Design review of the part built by this model. Coordinates are the model's own, in mm. A direction names the side the tool comes from. Round coordinates to 2 decimals unless told otherwise and drop trailing zeros. Order: outer loops, then holes, each group sorted by start corner. A loop starts at its lowest first (then second) coordinate and runs counter-clockwise, first axis right, second up. Notation, with made-up numbers: (39.5, 73) - (44.5, 73) arc R11 cw to (44.5, 93) - close; hole circle Ø4 at (89, 70). An arc over 180 degrees is marked (long way). Write item = value, one per line.
from build123d import *

# Parameters (mm, degrees)
SKETCH_1_W                = 380
SKETCH_1_H                = 270
EXTRUDE_1_DEPTH           = 7.5
CHAMFER_1_SIZE            = 1
SKETCH_2_R                = 20
CUT_EXTRUDE_1_DEPTH       = 15
HOLE_WIZARD_3_D           = 6.6
HOLE_WIZARD_3_CBORE_D     = 11
HOLE_WIZARD_3_CBORE_DEPTH = 6.8
SKETCH_9_R                = 5.5
CUT_EXTRUDE_2_DEPTH       = 234.559414283
SKETCH_11_R               = 52.5
CUT_EXTRUDE_3_DEPTH       = 4
HOLE_WIZARD_M6_1_D        = 5
SKETCH_15_R               = 3
CUT_EXTRUDE_4_DEPTH       = 9


with BuildPart() as part:
    # 草图1 → 凸台-拉伸1 (new, symmetric)
    with BuildSketch(Plane(origin=(0, 0, 0), x_dir=(1, 0, 0), z_dir=(0, 1, 0))):
        Rectangle(SKETCH_1_W, SKETCH_1_H)
    extrude(amount=EXTRUDE_1_DEPTH, both=True)

    # 倒角1
    chamfer_1_edges = [part.edges().sort_by_distance(p)[0] for p in [
        (190, 0, 135),
        (-190, 0, 135),
        (-190, 0, -135),
        (190, 0, -135),
    ]]
    chamfer(chamfer_1_edges, length=CHAMFER_1_SIZE)

    # 草图2 → 切除-拉伸1 (cut)
    with BuildSketch(Plane(origin=(0, 7.5, 0), x_dir=(1, 0, 0), z_dir=(0, 1, 0))):
        with Locations(Location((0, 0, 0), (0, 0, 270))):
            Circle(SKETCH_2_R)
    extrude(amount=-CUT_EXTRUDE_1_DEPTH, mode=Mode.SUBTRACT)

    # 打孔尺寸(%根据)内六角圆柱头螺钉的类型3 (through all)
    with Locations(Plane(origin=(0, 7.5, 0), x_dir=(1, 0, 0), z_dir=(0, 1, 0))):
        with Locations((-175, 120), (-60, 120), (-60, -120), (-175, 0), (-175, -120), (175, -120), (175, 0), (60, -120), (60, 120), (175, 120)):
            CounterBoreHole(HOLE_WIZARD_3_D / 2, HOLE_WIZARD_3_CBORE_D / 2, HOLE_WIZARD_3_CBORE_DEPTH)

    # 草图9 → 切除-拉伸2 (cut, through all)
    with BuildSketch(Plane(origin=(0, 7.5, 0), x_dir=(1, 0, 0), z_dir=(0, 1, 0))):
        with Locations(Location((-29.489473594, 20.648751709, 0), (0, 0, 270))):
            Circle(SKETCH_9_R)
        with Locations(Location((-29.489473594, -20.648751709, 0), (0, 0, 270))):
            Circle(SKETCH_9_R)
        with Locations(Location((-32.5, 0, 0), (0, 0, 270))):
            Circle(SKETCH_9_R)
        with Locations(Location((29.489473594, -20.648751709, 0), (0, 0, 90))):
            Circle(SKETCH_9_R)
        with Locations(Location((32.5, 0, 0), (0, 0, 90))):
            Circle(SKETCH_9_R)
        with Locations(Location((29.489473594, 20.648751709, 0), (0, 0, 90))):
            Circle(SKETCH_9_R)
    extrude(amount=-CUT_EXTRUDE_2_DEPTH, mode=Mode.SUBTRACT)

    # 草图11 → 切除-拉伸3 (cut)
    with BuildSketch(Plane(origin=(0, 7.5, 0), x_dir=(1, 0, 0), z_dir=(0, 1, 0))):
        with Locations(Location((0, 0, 0), (0, 0, 270))):
            Circle(SKETCH_11_R)
    extrude(amount=-CUT_EXTRUDE_3_DEPTH, mode=Mode.SUBTRACT)

    # M6 螺纹孔1 (through all)
    with Locations(Plane(origin=(0, 7.5, 0), x_dir=(1, 0, 0), z_dir=(0, 1, 0))):
        with Locations((122.5, -7), (122.5, 23), (-122.5, 23), (-122.5, -7)):
            Hole(HOLE_WIZARD_M6_1_D / 2)

    # 草图15 → 切除-拉伸4 (cut)
    with BuildSketch(Plane(origin=(0, 3.5, 0), x_dir=(1, 0, 0), z_dir=(0, 1, 0))):
        with Locations(Location((43, 0, 0), (0, 0, 270))):
            Circle(SKETCH_15_R)
    extrude(amount=-CUT_EXTRUDE_4_DEPTH, mode=Mode.SUBTRACT)


solid = part.part
1) The part is to be moulded in two halves that separate along X. For faces 1 (the flat face through (-3, -7.5, -32)), 2 (the flat face through (190, 0, 2)), 3 (the cylindrical face through (-175.716, 4.148, 114.547)), say which applies: released by +X, released by -X, zero draft, split by the parting line, or undercut.
Findings:
face_1 = zero draft
face_2 = released by +X
face_3 = undercut
2) To check wall thickness, follow L1, parallel to X at y = 2.5, z = -120; L2, parallel to X at y = -3.5, z = -120; L3, parallel to Z at x = 60, y = -2.75. State the ranges of each line that lie inside material, in increasing order. Write a range as from..to.
Findings:
L1 = -190..-180.5, -169.5..-65.5, -54.5..54.5, 65.5..169.5, 180.5..190
L2 = -190..-178.3, -171.7..-63.3, -56.7..56.7, 63.3..171.7, 178.3..190
L3 = -135..-123.3, -116.7..116.7, 123.3..135
3) Clearance check with flat-ended pins moving along their axes: pin 1 Ø4 at (x, z) = (175, 0) entering from -Y; pin 2 Ø3.5 at (x, z) = (43, 0) entering from +Y; pin 3 Ø14.5 at (x, z) = (29.49, 20.65) entering from +Y; pin 4 Ø3.5 at (x, z) = (173.5, -118) entering from +Y. State where each tip first meets the part, or that it passes through.
Findings:
pin_1 = through
pin_2 = -5.5
pin_3 = 3.5
pin_4 = 0.7
4) We need section A-A on x = -42. Write out the cut boundary in (y, z), and give its area (3 significant figures).
Findings:
outline = (-7.5, -135) - (7.5, -135) - (7.5, -31.5) - (3.5, -31.5) - (3.5, 31.5) - (7.5, 31.5) - (7.5, 135) - (-7.5, 135) - close
area = 3,800 mm^2
5) We need section B-B on y = -3.25. Give the number of separate pieces and of enclosed holes in the cut face, and give its area (3 significant figures).
Findings:
separate_pieces = 1
enclosed_holes = 22
area = 100,000 mm^2
6) For faces 4 (the cylindrical face through (59.284, 4.148, -125.453)), 5 (the flat face through (-3, 0, 135)), list the 3-axis set-ups (+Z, -Z, +X, -X, +Y, -Y) from which the entire face can be reached by the end or side of a thin tool; tool diameter is ignored.
Findings:
face_4 = +Y
face_5 = +Z, +X, -X, +Y, -Y
